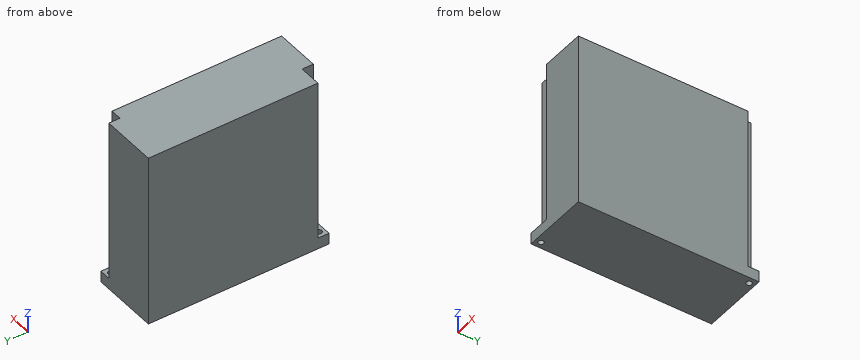
```python
from build123d import *

# Parameters (mm, degrees)
SKETCH1_W          = 60.2
SKETCH1_H          = 162
EXTRUDE1_DEPTH     = 155.9
SKETCH2_W          = 20
SKETCH2_H          = 10
SKETCH2_W_2        = 10
CUT_EXTRUDE1_DEPTH = 145.9
SKETCH3_R          = 2.5
CUT_EXTRUDE2_DEPTH = 179.246514692


with BuildPart() as part:
    # Sketch1 → Extrude1 (new body)
    with BuildSketch(Plane.XY):
        Rectangle(SKETCH1_W, SKETCH1_H)
    extrude(amount=EXTRUDE1_DEPTH)

    # Sketch2 → Cut-Extrude1 (cut)
    with BuildSketch(Plane.XY.offset(155.9)):
        with Locations((-20.1, -76)):
            Rectangle(SKETCH2_W, SKETCH2_H)
        with Locations((25.1, 76)):
            Rectangle(SKETCH2_W_2, SKETCH2_H)
    extrude(amount=-CUT_EXTRUDE1_DEPTH, mode=Mode.SUBTRACT)

    # Sketch3 → Cut-Extrude2 (cut, through all)
    with BuildSketch(Plane.XY.offset(155.9)):
        with Locations((24.5, 76)):
            Circle(SKETCH3_R)
        with Locations((-24.5, -76)):
            Circle(SKETCH3_R)
    extrude(amount=-CUT_EXTRUDE2_DEPTH, mode=Mode.SUBTRACT)


solid = part.part
```
Part model, mm, in its own coordinate system. Give positions to 0.01 mm unless a question says otherwise; leave off trailing zeros. Order: outer loops, then holes, each group sorted by start corner. A loop starts at its lowest first (then second) coordinate and runs counter-clockwise, first axis right, second up. Notation, with made-up numbers: M 6.25,81.5 L 12.25,81.5 A31 ccw 12.25,117.5 Z; hole C 24,68 d4. An arc over 180 degrees is marked long. Use a Markdown table: item, result. Add a question column.
(1) Saw through at C-C, the plane z = 31. Give the cut face in (x, y), and give its area (3 significant figures).
(2) Saw through at B-B, the plane x = -24.5. Give the cut face in (y, z).
(3) Saw through at D-D, the plane x = -16. Give the cut face in (y, z), and give its area (3 significant figures).
(4) Probe line 1 along Y through (x, z) = (24.5, 6); line 2 along Y through (x, z) = (-24.5, 7.75); line 3 along Y through (x, z) = (-16, 102). List the from-to ranges inside material, lowest first. Write a range as [from, to].
(5) Saw through at A-A, the plane y = 76. Give the cut face in (x, z).
(6) Drop flat-ended pins along their axis: P1, Ø3, axis at y = -78, z = 106.5, coming from the -X side; P2, Ø5, axis at y = 76, z = 100.5, coming from the +X side; P3, Ø22, axis at x = -22, z = 112, coming from the -Y side. Give the stop position or say it passes through.
Answer key:
| question | item | result |
|---|---|---|
| 1 | outline | M -30.1,-71 L -10.1,-71 L -10.1,-81 L 30.1,-81 L 30.1,71 L 20.1,71 L 20.1,81 L -30.1,81 Z |
| 1 | area | 9,450 mm^2 |
| 2 | outline | M -81,0 L -78.5,0 L -78.5,10 L -81,10 Z; M -73.5,0 L 81,0 L 81,155.9 L -71,155.9 L -71,10 L -73.5,10 Z |
| 3 | outline | M -81,0 L 81,0 L 81,155.9 L -71,155.9 L -71,10 L -81,10 Z |
| 3 | area | 23,800 mm^2 |
| 4 | line 1 | [-81, 73.5], [78.5, 81] |
| 4 | line 2 | [-81, -78.5], [-73.5, 81] |
| 4 | line 3 | [-71, 81] |
| 5 | outline | M -30.1,0 L 22,0 L 22,10 L 20.1,10 L 20.1,155.9 L -30.1,155.9 Z; M 27,0 L 30.1,0 L 30.1,10 L 27,10 Z |
| 6 | P1 | x = -10.1 |
| 6 | P2 | x = 20.1 |
| 6 | P3 | y = -71 |
